```python
from build123d import *

# Parameters (mm, degrees)
BOSS_EXTRUDE1_DEPTH = 2000
SHELL1_T            = -4


with BuildPart() as part:
    # Sketch1 → Boss-Extrude1 (new body)
    with BuildSketch(Plane.XY):
        with BuildLine():
            Line((41.8, 50), (-41.8, 50))
            ThreePointArc((-41.8, 50), (-47.598275606, 47.598275606), (-50, 41.8))
            Line((-50, 41.8), (-50, -41.8))
            ThreePointArc((-50, -41.8), (-47.598275606, -47.598275606), (-41.8, -50))
            Line((-41.8, -50), (41.8, -50))
            ThreePointArc((41.8, -50), (47.598275606, -47.598275606), (50, -41.8))
            Line((50, -41.8), (50, 41.8))
            ThreePointArc((50, 41.8), (47.598275606, 47.598275606), (41.8, 50))
        make_face()
    extrude(amount=BOSS_EXTRUDE1_DEPTH)

    # Shell1
    shell1_openings = [part.faces().sort_by_distance(p)[0] for p in [
        (0, 0, 2000),
        (0, 0, 0),
    ]]
    offset(amount=SHELL1_T, openings=shell1_openings, kind=Kind.INTERSECTION)


solid = part.part
```
Read the model definition and answer for the solid it produces. Units are mm, in the model's axes. A direction names the side the tool comes from. Coordinates: 2 decimals unless noted, no trailing zeros. Loops run counter-clockwise (first coordinate to the right, second up) from the corner with the lowest first, then second, coordinate; pieces in that order, holes last. Notation, with made-up numbers: (71, -25) - (107, -25) arc R16 ccw to (107, -6) - close; hole circle Ø9 at (6, 11.25). An arc over 180 degrees is marked (long way). Answer in a Markdown table with one row per item.
1. Which of the six approach directions +Z, -Z, +X, -X, +Y, -Y give full straight-line access (tool end or side, diameter ignored) to faces 5 (the face through (1, 50, 986)), 6 (the face through (-1, -46, 986))?
Conclusion:
| item | result |
|---|---|
| face 5 | +Z, -Z, +X, -X, +Y |
| face 6 | +Z, -Z |
2. Find section B-B, the plane z = 957.5. Write down the section's boundary in (x, y).
Conclusion:
| item | result |
|---|---|
| outline | (-50, -41.8) arc R8.2 ccw to (-41.8, -50) - (41.8, -50) arc R8.2 ccw to (50, -41.8) - (50, 41.8) arc R8.2 ccw to (41.8, 50) - (-41.8, 50) arc R8.2 ccw to (-50, 41.8) - close; hole (-46, -41.8) arc R4.2 ccw to (-41.8, -46) - (41.8, -46) arc R4.2 ccw to (46, -41.8) - (46, 41.8) arc R4.2 ccw to (41.8, 46) - (-41.8, 46) arc R4.2 ccw to (-46, 41.8) - close |
3. Determine the mould class of faces 1 (the face through (50, -1, 986)), 2 (the face through (1, 46, 986)), 3 (the face through (-50, 1, 986)), 4 (the face through (-1, -50, 986)) for opening direction X: +X half, -X half, draft (parallel to the pull), parting line (faces both ways), or undercut.
Conclusion:
| item | result |
|---|---|
| face 1 | +X half |
| face 2 | undercut |
| face 3 | -X half |
| face 4 | draft |
4. Straight lines are drawn through the part: line 1 (X direction, y = 25.5, z = 264.5); line 2 (Y direction, x = 42.5, z = 462). For each, find the intervals that lie inside material, in ascending order.
Conclusion:
| item | result |
|---|---|
| line 1 | x = -50 to -46, 46 to 50 |
| line 2 | y = -49.97 to -45.94, 45.94 to 49.97 |
5. Find section A-A, the plane x = -26. Write down the section's boundary in (y, z), then the cut area to 3 significant figures.
Conclusion:
| item | result |
|---|---|
| outline | (-50, 0) - (-46, 0) - (-46, 2000) - (-50, 2000) - close; (46, 0) - (50, 0) - (50, 2000) - (46, 2000) - close |
| area | 16,000 mm² |
